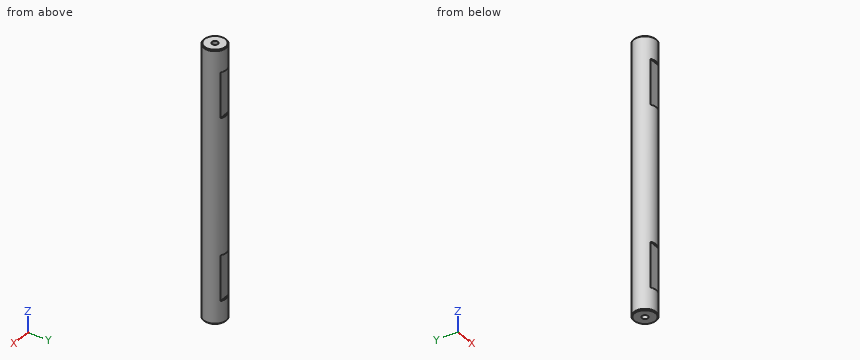
```python
from build123d import *

# Parameters (mm, degrees)
SKETCH_1_R          = 12.5
EXTRUDE_1_DEPTH     = 150
SKETCH_2_W          = 50
SKETCH_2_H          = 2
CUT_EXTRUDE_1_DEPTH = 100
CHAMFER_1_SIZE      = 1


with BuildPart() as part:
    # 草图1 → 凸台-拉伸1 (new, symmetric)
    with BuildSketch(Plane.XY):
        Circle(SKETCH_1_R)
    extrude(amount=EXTRUDE_1_DEPTH, both=True)

    # 草图2 → 切除-拉伸1 (cut, symmetric)
    with BuildSketch(Plane(origin=(0, 0, 0), x_dir=(0, 0, -1), z_dir=(1, 0, 0))):
        with Locations((-100, 11.5)):
            Rectangle(SKETCH_2_W, SKETCH_2_H)
        with Locations((-100, -11.5)):
            Rectangle(SKETCH_2_W, SKETCH_2_H)
        with Locations((100, -11.5)):
            Rectangle(SKETCH_2_W, SKETCH_2_H)
        with Locations((100, 11.5)):
            Rectangle(SKETCH_2_W, SKETCH_2_H)
    extrude(amount=CUT_EXTRUDE_1_DEPTH, both=True, mode=Mode.SUBTRACT)

    # 倒角1
    chamfer_1_edges = [part.edges().sort_by_distance(p)[0] for p in [
        (-12.5, 0, -150),
        (-12.5, 0, 150),
    ]]
    chamfer(chamfer_1_edges, length=CHAMFER_1_SIZE)

    # 草图4 → M8 螺纹孔1 (revolve, cut)
    with BuildSketch(Plane(origin=(0, 0, -150), x_dir=(0, 1, 0), z_dir=(1, 0, 0))):
        Polygon((0, 0), (0, 21.792926105), (3.4, 19.75), (3.4, 0), align=None)
    hole_wizard_m8_1 = revolve(axis=Axis((0, 0, -156.35), (0, 0, 1)), mode=Mode.SUBTRACT)

    # 镜向1: M8 螺纹孔1 across plane
    add(hole_wizard_m8_1.mirror(Plane.XY), mode=Mode.SUBTRACT)


solid = part.part
```
Work out the finished part from the listing and answer in its coordinate system (mm). Give positions to 0.01 mm unless a question says otherwise; leave off trailing zeros. Order: outer loops, then holes, each group sorted by start corner. A loop starts at its lowest first (then second) coordinate and runs counter-clockwise, first axis right, second up.
1. Section B-B, the plane z = 122 is taken. Determine the outline of the cut face in (x, y).
Result sheet:
outline: (-6.78, -10.5) - (6.78, -10.5) arc R12.5 ccw to (6.78, 10.5) - (-6.78, 10.5) arc R12.5 ccw to start
2. Each of these flat-tipped pins is pushed along its axis until it touches: P1, Ø0.6, axis at x = -0.5, y = -12, coming from the -Z side; P2, Ø0.6, axis at x = -1.5, y = 12, coming from the +Z side; P3, Ø1.5, axis at y = -6.5, z = 51.5, coming from the +X side. Where does it stop, or does it pass through?
Result sheet:
P1: stops at z = -149.79
P2: stops at z = 149.71
P3: stops at x = 11.1
3. Straight lines are drawn through the part: L1, parallel to Y at x = 0, z = -138.5; L2, parallel to Y at x = 0.75, z = 4.5; L3, parallel to X at y = -10.5, z = -39.5. For each, find the intervals that lie inside material, in ascending order.
Result sheet:
L1: y = -12.5 to -3.4, 3.4 to 12.5
L2: y = -12.48 to 12.48
L3: x = -6.78 to 6.78
4. Section A-A, the plane z = -50 is taken. Determine the outline of the cut face in (x, y), and give its area (3 significant figures).
Result sheet:
outline: circle Ø25 at (0, 0)
area: 491 mm2
